Part model, mm, in its own coordinate system. Face numbers are marked on the shaded views. A direction names the side the tool comes from. Coordinates: 2 decimals unless noted, no trailing zeros. Write each loop counter-clockwise with the first axis right and the second up, starting at its lowest first coordinate (ties: lowest second). Pieces come first, ordered by that corner, then holes. Notation, with made-up numbers: M 60.25,36.5 L 104.25,36.5 A25 cw 104.25,59.5 Z; hole C -18.75,-35.75 d7. An arc over 180 degrees is marked long. Use a Markdown table: item, result. Add a question column.
Q1. Slice it at C-C on y = 10. Write the cut outline in (x, z).
Q2. Mould opens along X. For the marked faces 3, 4 and 5 say: released by +X, released by -X, zero draft, split by the parting line, or undercut.
Q3. Wall check: L1, parallel to Y at x = 2.75, z = 6.25; L2, parallel to Y at x = -6, z = 5; L3, parallel to Y at x = -7.25, z = 2.5. Give the ranges that are in metal, low to high. Write a range as from..to.
Q4. Pin check, flat tips, straight feed: pin 1 Ø6 at (y, z) = (7.5, 6.5) entering from +X; pin 2 Ø5 at (y, z) = (8.5, 0.5) entering from +X; pin 3 Ø6 at (y, z) = (17, -5) entering from -X. Stop position of each tip, or through.
Q5. Slice it at B-B on y = 3. Write the cut outline in (x, z).
Q6. Tool access for the marked faces 1 and 2: list every direction of +Z, -Z, +X, -X, +Y, -Y with a clear straight run to the whole face (end or side of a thin tool).
Q7. Slice it at A-A on y = 22. Write the cut outline in (x, z).
from build123d import *

# Parameters (mm, degrees)
SIDE_CUT_A_8_DEPTH      = 4
SIDE_CUT_A_8_DEPTH_BACK = 14
SIDE_CUT_A_8_SKETCH_R   = 4
SIDE_CUT_B_8_DEPTH      = 4
SIDE_CUT_B_8_DEPTH_BACK = 14
SIDE_CUT_B_8_SKETCH_R   = 4


with BuildPart() as part:
    # Knob Profile Sketch → Knob Body Revolve (revolve)
    with BuildSketch(Plane.XY, mode=Mode.PRIVATE) as knob_body_revolve_sk:
        with BuildLine():
            Line((0, 24), (0, 0))
            Line((0, 0), (7, 0))
            Line((7, 0), (7, 4.013980889))
            ThreePointArc((7, 4.013980889), (6.494199283, 6.419547181), (7.490711985, 8.666666667))
            ThreePointArc((7.490711985, 8.666666667), (7.999225249, 10.055663319), (7.414213562, 11.414213562))
            ThreePointArc((7.414213562, 11.414213562), (6.243817658, 14.14561297), (7.28036451, 16.930561789))
            ThreePointArc((7.28036451, 16.930561789), (7.34643685, 17.001626612), (7.414213562, 17.071067812))
            ThreePointArc((7.414213562, 17.071067812), (9.308465087, 28.041428182), (0, 34.147938905))
            Line((0, 34.147938905), (0, 24))
        make_face()
    revolve(knob_body_revolve_sk.sketch.rotate(Axis((0, 0, 0), (0, 1, 0)), 90), axis=Axis((0, 0, 0), (0, 1, 0)))

    # Side Cut A Ø8 Sketch → Side Cut A Ø8 (cut, two sides: drawn at the far end of the back side and taken through both)
    with BuildSketch(Plane.XY.offset(-SIDE_CUT_A_8_DEPTH_BACK)):
        with Locations((0, 24)):
            Circle(SIDE_CUT_A_8_SKETCH_R)
    extrude(amount=SIDE_CUT_A_8_DEPTH + SIDE_CUT_A_8_DEPTH_BACK, mode=Mode.SUBTRACT)

    # Side Cut B Ø8 Sketch → Side Cut B Ø8 (cut, two sides: drawn at the far end of the back side and taken through both)
    with BuildSketch(Plane(origin=(0, 0, 0), x_dir=(0, 0, -1), z_dir=(1, 0, 0)).offset(-SIDE_CUT_B_8_DEPTH_BACK)):
        with Locations(Location((0, 24, 0), (0, 0, 180))):
            Circle(SIDE_CUT_B_8_SKETCH_R)
    extrude(amount=SIDE_CUT_B_8_DEPTH + SIDE_CUT_B_8_DEPTH_BACK, mode=Mode.SUBTRACT)


solid = part.part
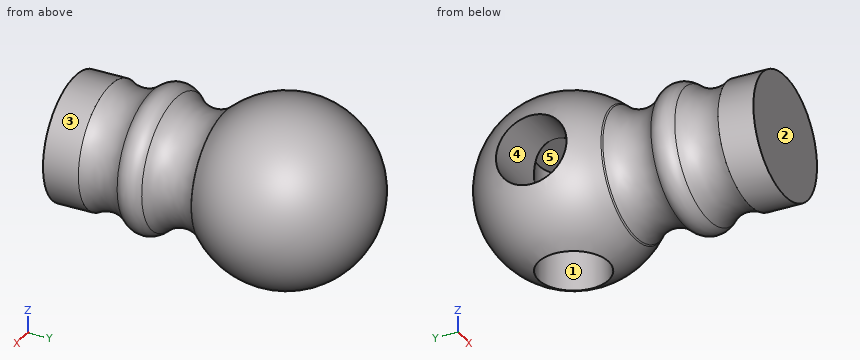
Recorded:
| question | item | result |
|---|---|---|
| 1 | outline | C 0,0 d16 |
| 2 | face 3 | split by the parting line |
| 2 | face 4 | zero draft |
| 2 | face 5 | undercut |
| 3 | L1 | 0..4.35, 7.65..12.16, 16.33..31.51 |
| 3 | L2 | 9.15..10.85, 17.52..30.48 |
| 3 | L3 | 8.9..11.1, 17.35..20.88, 27.12..30.65 |
| 4 | pin 1 | x = 6.72 |
| 4 | pin 2 | x = 8 |
| 4 | pin 3 | x = -8.46 |
| 5 | outline | C 0,0 d14 |
| 6 | face 1 | -Z |
| 6 | face 2 | +Z, -Z, +X, -X, -Y |
| 7 | outline | M -9.33,-3.46 A9.95 ccw -3.46,-9.33 L -3.46,-3.46 Z; M -9.33,3.46 L -3.46,3.46 L -3.46,4 L 3.46,4 L 3.46,3.46 L 4,3.46 L 4,-3.46 L 3.46,-3.46 L 3.46,-9.33 A9.95 ccw long Z |
